Check sheet for the modelled part. Datum: model origin and axes. Units: mm. Coordinates: 2 decimals unless noted, no trailing zeros. Loops run counter-clockwise (first coordinate to the right, second up) from the corner with the lowest first, then second, coordinate; pieces in that order, holes last.
```python
from build123d import *

# Parameters (mm, degrees)
SKETCH1_W           = 108.732266051
SKETCH1_H           = 21.168090093
SKETCH1_R           = 5
BOSS_EXTRUDE1_DEPTH = 4.5


with BuildPart() as part:
    # Sketch1 → Boss-Extrude1 (new body)
    with BuildSketch(Plane(origin=(0, 0, 0), x_dir=(1, 0, 0), z_dir=(0, 1, 0))):
        with Locations((54.366133026, 10.584045046)):
            Rectangle(SKETCH1_W, SKETCH1_H)
        with Locations(Location((54.366133025, 10.584045046, 0), (0, 0, 270))):
            Circle(SKETCH1_R, mode=Mode.SUBTRACT)
    extrude(amount=BOSS_EXTRUDE1_DEPTH)


solid = part.part
```
1) Section check B-B on z = -12. Enter the section's corners in (x, y), plus the area to 3 significant figures.
Answer sheet:
outline: (0, 0) - (49.57, 0) - (49.57, 4.5) - (0, 4.5) - close; (59.16, 0) - (108.73, 0) - (108.73, 4.5) - (59.16, 4.5) - close
area: 446 mm2
2) Section check C-C on y = 0.95. Enter the section's corners in (x, z), plus the area to 3 significant figures.
Answer sheet:
outline: (0, -21.17) - (108.73, -21.17) - (108.73, 0) - (0, 0) - close; hole circle Ø10 at (54.37, -10.58)
area: 2,220 mm2
3) Depth check by flat-ended pin: pin 1 (9 mm diameter, centred on x = 54.37, z = -10.58, fed in from -Y). Enter the tip coordinate at first touch or a pass-through.
Answer sheet:
pin 1: passes through
4) Scan lines: line 1 (X direction, y = 3.55, z = -11); line 2 (Z direction, x = 53.5, y = 2.05). Record each from-to range of solid material in increasing order.
Answer sheet:
line 1: x = 0 to 49.38, 59.35 to 108.73
line 2: z = -21.17 to -15.51, -5.66 to 0
5) Section check A-A on x = 52. Enter the section's corners in (y, z).
Answer sheet:
outline: (0, -21.17) - (4.5, -21.17) - (4.5, -14.99) - (0, -14.99) - close; (0, -6.18) - (4.5, -6.18) - (4.5, 0) - (0, 0) - close
6) Mould release check, pull along Z, two halves, no side actions. Record for faces 1 (the flat face through (54, 2, -21.168)), 2 (the flat face through (54, 0, -4)), 3 (the cylindrical face through (59.324, 2.218, -11.235)), 4 (the flat face through (54, 2, 0)): +Z half, -Z half, draft (parallel to the pull), parting line (faces both ways), or undercut.
Answer sheet:
face 1: -Z half
face 2: draft
face 3: undercut
face 4: +Z half
